Can you work these out from the model? Positions are in its coordinate system, mm. A direction names the side the tool comes from. Coordinates: 2 decimals unless noted, no trailing zeros. Write each loop counter-clockwise with the first axis right and the second up, starting at its lowest first coordinate (ties: lowest second). Pieces come first, ordered by that corner, then holes.
```python
from build123d import *

# Parameters (mm, degrees)
EXTRUDE_1_DEPTH = 800


with BuildPart() as part:
    # 草图1 → 拉伸-薄壁1 (new body)
    with BuildSketch(Plane.XY):
        with BuildLine():
            Line((450, -74.939443754), (-450, -74.939443754))
            ThreePointArc((-450, -74.939443754), (-530, 5.060556246), (-450, 85.060556246))
            Line((-450, 85.060556246), (450, 85.060556246))
            ThreePointArc((450, 85.060556246), (530, 5.060556246), (450, -74.939443754))
        make_face()
        with BuildLine():
            Line((450, -69.939443754), (-450, -69.939443754))
            ThreePointArc((-450, -69.939443754), (-525, 5.060556246), (-450, 80.060556246))
            Line((-450, 80.060556246), (450, 80.060556246))
            ThreePointArc((450, 80.060556246), (525, 5.060556246), (450, -69.939443754))
        make_face(mode=Mode.SUBTRACT)
    extrude(amount=EXTRUDE_1_DEPTH)


solid = part.part
```
1. Which directions (+Z, -Z, +X, -X, +Y, -Y) give clear straight access to the entire face, cutting with the end or side of a thin tool? Please do faces 1 (the face through (-529.98, 3.3, 394.4)), 2 (the face through (524.98, 6.71, 394.4)).
2. If I drill on L1, parallel to X at y = 4.5, z = 757; L2, parallel to Y at x = -195, z = 274; L3, parallel to X at y = -2, z = 243.5, over which ranges is the centre line in solid material (lowest first)?
3. If we section it at B-B, the plane y = -3: List the corners of the cut face in (x, z) for me, plus the area to 3 significant figures.
4. We'd pull the mould along Y, two halves only. Please class faces 3 (the face through (529.98, 6.82, 394.4)), 4 (the face through (-6, 80.061, 394)), 5 (the face through (2, 82, 800)): released by +Y, released by -Y, zero draft, split by the parting line, or undercut.
5. If we section it at C-C, the plane z = 724: List the corners of the cut face in (x, y) for me, plus the area to 3 significant figures.
6. I'm going to push flat-ended pins straight in: P1, Ø1.5, axis at y = -9, z = 207, coming from the -X side; P2, Ø10, axis at y = 46, z = 398.5, coming from the +X side; P3, Ø2, axis at y = -33.5, z = 255.5, coming from the +X side. Where does each tip first touch, or does it pass through?
7. If we section it at A-A, the plane x = -153: List the corners of the cut face in (y, z) for me, plus the area to 3 significant figures.
Answers:
1. face 1: +Z, -Z, -X
1. face 2: +Z, -Z
2. L1: x = -530 to -525, 525 to 530
2. L2: y = -74.94 to -69.94, 80.06 to 85.06
2. L3: x = -529.69 to -524.67, 524.67 to 529.69
3. outline: (-529.59, 0) - (-524.57, 0) - (-524.57, 800) - (-529.59, 800) - close; (524.57, 0) - (529.59, 0) - (529.59, 800) - (524.57, 800) - close
3. area: 8,040 mm2
4. face 3: split by the parting line
4. face 4: undercut
4. face 5: zero draft
5. outline: (-450, -74.94) - (450, -74.94) arc R80 ccw to (450, 85.06) - (-450, 85.06) arc R80 ccw to start; hole (-450, -69.94) - (450, -69.94) arc R75 ccw to (450, 80.06) - (-450, 80.06) arc R75 ccw to start
5. area: 11,400 mm2
6. P1: stops at x = -528.88
6. P2: stops at x = 521.47
6. P3: stops at x = 520.63
7. outline: (-74.94, 0) - (-69.94, 0) - (-69.94, 800) - (-74.94, 800) - close; (80.06, 0) - (85.06, 0) - (85.06, 800) - (80.06, 800) - close
7. area: 8,000 mm2
